```python
from build123d import *

# Parameters (mm, degrees)
SKETCH_1_R               = 7
EXTRUDE_1_DEPTH          = 357.5
CHAMFER_1_SIZE           = 0.5
CUT_EXTRUDE_1_DEPTH      = 358.637036673
CUT_EXTRUDE_1_DEPTH_BACK = 358.637036673


with BuildPart() as part:
    # 草图1 → 凸台-拉伸1 (new, symmetric)
    with BuildSketch(Plane(origin=(0, 0, 0), x_dir=(1, 0, 0), z_dir=(0, 1, 0))):
        with Locations(Location((0, 0, 0), (0, 0, 270))):
            Circle(SKETCH_1_R)
    extrude(amount=EXTRUDE_1_DEPTH, both=True)

    # 倒角1
    chamfer_1_edges = [part.edges().sort_by_distance(p)[0] for p in [
        (0, -357.5, -7),
        (0, 357.5, -7),
    ]]
    chamfer(chamfer_1_edges, length=CHAMFER_1_SIZE)

    # 草图2 → 切除-拉伸1 (cut, two sides: drawn at the far end of the back side and taken through both)
    with BuildSketch(Plane(origin=(0, 0, 0), x_dir=(0, 0, -1), z_dir=(1, 0, 0)).offset(-CUT_EXTRUDE_1_DEPTH_BACK)):
        with BuildLine():
            Line((-3, -351.5), (-3, -348.5))
            ThreePointArc((-3, -348.5), (0, -345.5), (3, -348.5))
            Line((3, -348.5), (3, -351.5))
            ThreePointArc((3, -351.5), (0, -354.5), (-3, -351.5))
        make_face()
        with BuildLine():
            Line((-3, 351.5), (-3, 348.5))
            ThreePointArc((-3, 348.5), (0, 345.5), (3, 348.5))
            Line((3, 348.5), (3, 351.5))
            ThreePointArc((3, 351.5), (0, 354.5), (-3, 351.5))
        make_face()
    extrude(amount=CUT_EXTRUDE_1_DEPTH + CUT_EXTRUDE_1_DEPTH_BACK, mode=Mode.SUBTRACT)


solid = part.part
```
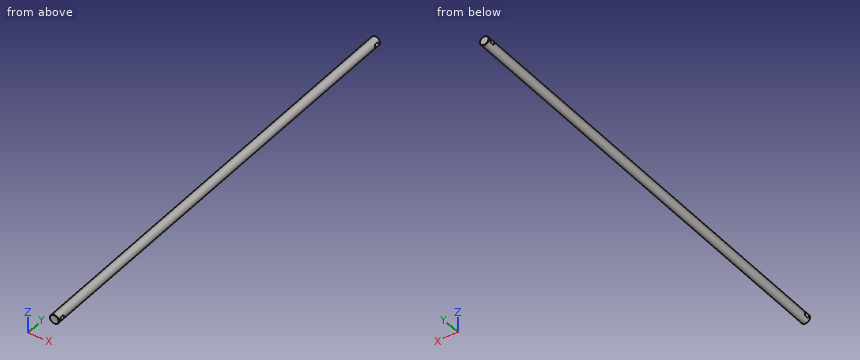
Geometry: final body of the model. Coordinates: model frame, mm. Give positions to 0.01 mm unless a question says otherwise; leave off trailing zeros. Loops run counter-clockwise (first coordinate to the right, second up) from the corner with the lowest first, then second, coordinate; pieces in that order, holes last. Notation, with made-up numbers: (23, 34.5) -> (34, 34.5) arc R23 cw to (34, 62.5) -> close; hole circle Ø7 at (24, 42). An arc over 180 degrees is marked (long way). Use CSV: the item, a comma, the result in double quotes.
(1) Cut plane C-C (y = -218.5). Output: boundary loops of the cut face in (x, z), plus the area to 3 significant figures.
From the geometry:
outline,"circle Ø14 at (0, 0)"
area,"154 mm^2"
(2) Cut plane A-A (z = 0). Output: boundary loops of the cut face in (x, y), plus the area to 3 significant figures.
From the geometry:
outline,"(-7, -357) -> (-6.5, -357.5) -> (6.5, -357.5) -> (7, -357) -> (7, -354.5) -> (-7, -354.5) -> close; (-7, -345.5) -> (7, -345.5) -> (7, 345.5) -> (-7, 345.5) -> close; (-7, 354.5) -> (7, 354.5) -> (7, 357) -> (6.5, 357.5) -> (-6.5, 357.5) -> (-7, 357) -> close"
area,"9,760 mm^2"
(3) Cut plane B-B (x = -3.75). Count the separate pieces of the cut face and the enclosed holes in it, plus the area to 3 significant figures.
From the geometry:
separate pieces,"1"
enclosed holes,"2"
area,"8,360 mm^2"
(4) Ray query, line 1 along Y through (x, z) = (-4, 0.25); line 2 along Y through (x, z) = (-0.75, -1); line 3 along X through (y, z) = (63.5, -2.25). Return the intervals inside material, ascending. Write a range as [from, to].
From the geometry:
line 1,"[-357.5, -354.49], [-345.51, 345.51], [354.49, 357.5]"
line 2,"[-357.5, -354.33], [-345.67, 345.67], [354.33, 357.5]"
line 3,"[-6.63, 6.63]"
(5) First-contact query: P1, Ø5, axis at x = -5, y = 45, coming from the +Z side; P2, Ø3.5, axis at x = 3, y = -350, coming from the +Z side; P3, Ø3.5, axis at x = -2.5, y = -350.5, coming from the -Z side. Flat tips, straight axial feed; report the tip coordinate or a pass-through.
From the geometry:
P1,"z = 6.54"
P2,"z = 6.89"
P3,"z = -6.96"
